Verification items for this drawing (mm, ordinates from the low corner). A direction names the side the tool comes from. Round coordinates to 2 decimals unless told otherwise and drop trailing zeros. Loops run counter-clockwise (first coordinate to the right, second up) from the corner with the lowest first, then second, coordinate; pieces in that order, holes last. Notation, with made-up numbers: (-9.75, 55.5) - (5.25, 55.5) arc R23 cw to (5.25, 76.5) - close; hole circle Ø4 at (19.5, -36.75). An arc over 180 degrees is marked (long way). Answer in a Markdown table with one row per item. Add a question column.
(1) Cross-section at C-C on x = 33.5. Enter the section's corners in (y, z), then the cut area to 3 significant figures.
(2) Cross-section at A-A on y = 13. Enter the section's corners in (x, z), then the cut area to 4 significant figures.
(3) Cross-section at D-D on z = 23.5. Enter the section's corners in (x, y), then the cut area to 3 significant figures.
(4) Gauge pin test, flat ends, axial feed: pin 1 (10 mm diameter, centred on x = 50, y = 18.5, fed in from -Z); pin 2 (4 mm diameter, centred on x = 62.5, z = 11.5, fed in from +Y); pin 3 (5 mm diameter, centred on x = 8, z = 19.5, fed in from -Y). Record the tip position at first contact, or that the pin passes through.
(5) Thickness scan on line 1 along X through (y, z) = (20.25, 10.5); line 2 along X through (y, z) = (23, 8.75); line 3 along Z through (x, y) = (61.5, 7.5). Record the ranges inside material, lowest first.
(6) Access from +Z, -Z, +X, -X, +Y, -Y to the whole of each face (thin tool, end or side, straight path). Record for the marked faces 1 and 2.
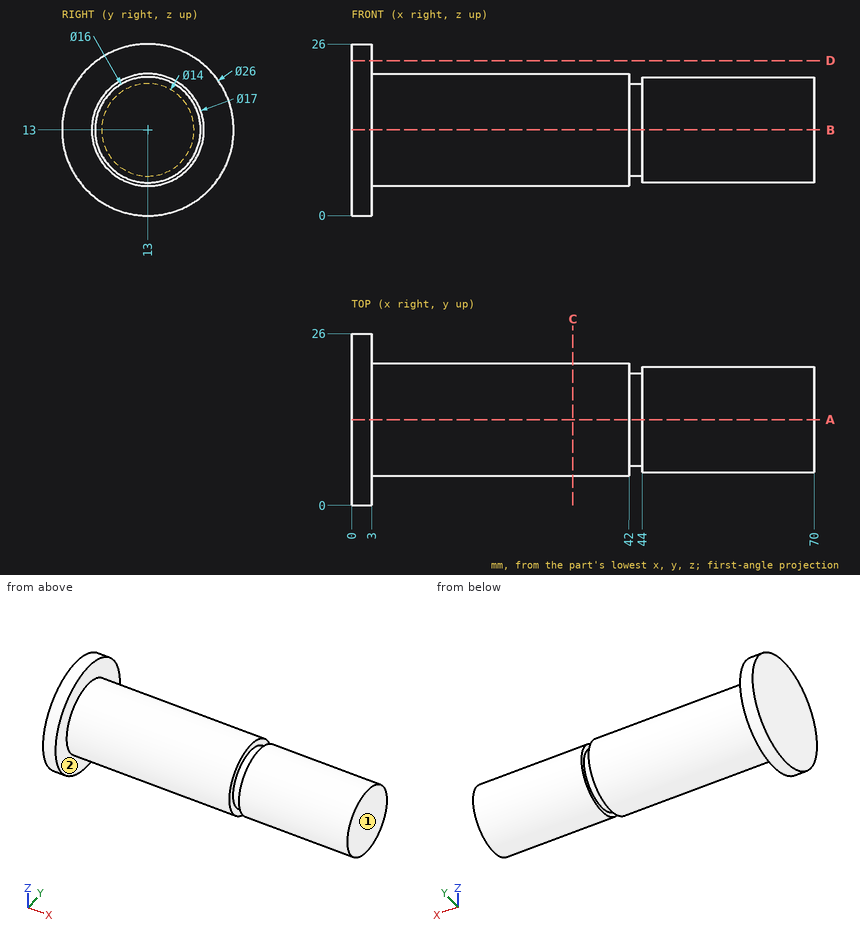
Answers:
| question | item | result |
|---|---|---|
| 1 | outline | circle Ø17 at (13, 13) |
| 1 | area | 227 mm^2 |
| 2 | outline | (0, 0) - (3, 0) - (3, 4.5) - (42, 4.5) - (42, 6) - (44, 6) - (44, 5) - (70, 5) - (70, 21) - (44, 21) - (44, 20) - (42, 20) - (42, 21.5) - (3, 21.5) - (3, 26) - (0, 26) - close |
| 2 | area | 1,185 mm^2 |
| 3 | outline | (0, 5.34) - (3, 5.34) - (3, 20.66) - (0, 20.66) - close |
| 3 | area | 46.0 mm^2 |
| 4 | pin 1 | stops at z = 5.02 |
| 4 | pin 2 | stops at y = 21 |
| 4 | pin 3 | stops at y = 5.5 |
| 5 | line 1 | x = 0 to 42, 44 to 70 |
| 5 | line 2 | x = 0 to 3 |
| 5 | line 3 | z = 7.19 to 18.81 |
| 6 | face 1 | +Z, -Z, +X, +Y, -Y |
| 6 | face 2 | +X |
